Can you work these out from the model? Positions are in its coordinate system, mm. A direction names the side the tool comes from. Give positions to 0.01 mm unless a question says otherwise; leave off trailing zeros. Write each loop counter-clockwise with the first axis right and the second up, starting at its lowest first coordinate (ties: lowest second). Pieces come first, ordered by that corner, then holes.
from build123d import *

# Parameters (mm, degrees)
SKETCH_1_W          = 60
SKETCH_1_H          = 60
EXTRUDE_1_DEPTH     = 60
SKETCH_3_R          = 4
EXTRUDE_2_DEPTH     = 12
SKETCH_4_W          = 60
SKETCH_4_H          = 60
SKETCH_4_W_2        = 58
SKETCH_4_H_2        = 58
CUT_EXTRUDE_4_DEPTH = 7
FILLET_4_R          = 5
CHAMFER_1_SIZE      = 1
FILLET_6_R          = 5
SKETCH_7_W          = 28
SKETCH_7_H          = 38
EXTRUDE_3_DEPTH     = 24
SKETCH_8_W          = 44.228024
SKETCH_8_H          = 29.89004
SKETCH_8_R          = 7
CUT_EXTRUDE_5_DEPTH = 4


with BuildPart() as part:
    # 草图1 → 凸台-拉伸1 (new body)
    with BuildSketch(Plane.XY):
        Rectangle(SKETCH_1_W, SKETCH_1_H)
    extrude(amount=EXTRUDE_1_DEPTH)

    # 草图3 → 凸台-拉伸2 (add)
    with BuildSketch(Plane.XY.offset(60)):
        Circle(SKETCH_3_R)
    extrude(amount=EXTRUDE_2_DEPTH)

    # 草图4 → 切除-拉伸4 (cut)
    with BuildSketch(Plane(origin=(0, 0, 0), x_dir=(-1, 0, 0), z_dir=(0, 0, -1))):
        Rectangle(SKETCH_4_W, SKETCH_4_H)
        Rectangle(SKETCH_4_W_2, SKETCH_4_H_2, mode=Mode.SUBTRACT)
    extrude(amount=-CUT_EXTRUDE_4_DEPTH, mode=Mode.SUBTRACT)

    # 圆角4
    fillet_4_edges = [part.edges().sort_by_distance(p)[0] for p in [
        (-29, -29, 3.5),
        (29, -29, 3.5),
        (29, 29, 3.5),
        (-29, 29, 3.5),
    ]]
    fillet(fillet_4_edges, radius=FILLET_4_R)

    # 倒角1
    chamfer_1_edges = [part.edges().sort_by_distance(p)[0] for p in [
        (0, 29, 0),
        (-29, 0, 0),
        (29, 0, 0),
        (0, -29, 0),
        (27.535533906, -27.535533906, 0),
        (-27.535533906, -27.535533906, 0),
        (-27.535533906, 27.535533906, 0),
        (27.535533906, 27.535533906, 0),
    ]]
    chamfer(chamfer_1_edges, length=CHAMFER_1_SIZE)

    # 圆角6
    fillet_6_edges = [part.edges().sort_by_distance(p)[0] for p in [
        (30, -30, 33.5),
        (-30, -30, 33.5),
        (-30, 30, 33.5),
        (30, 30, 33.5),
    ]]
    fillet(fillet_6_edges, radius=FILLET_6_R)

    # 草图7 → 凸台-拉伸3 (add)
    with BuildSketch(Plane(origin=(0, 30, 0), x_dir=(1, 0, 0), z_dir=(0, 1, 0))):
        with Locations((0, -38)):
            Rectangle(SKETCH_7_W, SKETCH_7_H)
    extrude(amount=EXTRUDE_3_DEPTH)

    # 草图8 → 切除-拉伸5 (cut)
    with BuildSketch(Plane(origin=(0, 0, 19), x_dir=(-1, 0, 0), z_dir=(0, 0, -1))):
        with Locations((0, 44.94502)):
            Rectangle(SKETCH_8_W, SKETCH_8_H)
        with Locations((0, 44.94502)):
            Circle(SKETCH_8_R, mode=Mode.SUBTRACT)
    extrude(amount=-CUT_EXTRUDE_5_DEPTH, mode=Mode.SUBTRACT)


solid = part.part
(1) Imagine slicing it at C-C, the plane y = -21. Write out the boundary of the cut face in (x, z).
Returned:
outline: (-30, 7) - (-29, 7) - (-29, 1) - (-28, 0) - (28, 0) - (29, 1) - (29, 7) - (30, 7) - (30, 60) - (-30, 60) - close
(2) For faces 4 (the face through (27, -28, 4)), 5 (the face through (-0.867, -3.905, 65.916)), 6 (the face through (27, 28, 4)), which set-ups out of +Z, -Z, +X, -X, +Y, -Y let a thin tool reach every point of the face, with its end or its side?
Returned:
face 4: -Z, +X, -Y
face 5: +Z
face 6: -Z, +X, +Y
(3) Will these pins go through, and if not, where does the flat tip stop? P1, Ø4, axis at x = 6, y = 14.5, coming from the +Z side; P2, Ø12, axis at x = 7.5, z = 10, coming from the +Y side; P3, Ø3, axis at x = 4.5, y = 35, coming from the -Z side; P4, Ø4, axis at x = 16.5, y = 39, coming from the -Z side.
Returned:
P1: stops at z = 60
P2: stops at y = 30
P3: stops at z = 23
P4: passes through
(4) Imagine slicing it at D-D, the plane z = 45. Write out the boundary of the cut face in (x, y), plus the area to 3 significant figures.
Returned:
outline: (-30, -25) arc R5 ccw to (-25, -30) - (25, -30) arc R5 ccw to (30, -25) - (30, 25) arc R5 ccw to (25, 30) - (14, 30) - (14, 54) - (-14, 54) - (-14, 30) - (-25, 30) arc R5 ccw to (-30, 25) - close
area: 4,250 mm2
(5) Imagine slicing it at A-A, the plane x = 0. Write out the boundary of the cut face in (y, z).
Returned:
outline: (-30, 7) - (-29, 7) - (-29, 1) - (-28, 0) - (28, 0) - (29, 1) - (29, 7) - (30, 7) - (30, 23) - (37.95, 23) - (37.95, 19) - (51.95, 19) - (51.95, 23) - (54, 23) - (54, 57) - (30, 57) - (30, 60) - (4, 60) - (4, 72) - (-4, 72) - (-4, 60) - (-30, 60) - close
(6) If we mould it in two halves opening along Y, with no side actions, what happens to faces 1 (the face through (-14, 42, 40)), 2 (the face through (29, 28, 34)), 3 (the face through (-6.466, 42.264, 20.972))? For each: +Y half, -Y half, draft (parallel to the pull), parting line (faces both ways), or undercut.
Returned:
face 1: draft
face 2: +Y half
face 3: undercut
(7) If I drill on L1, parallel to X at y = 41.5, z = 36; L2, parallel to Z at x = -24, y = -10; L3, parallel to X at y = 21.5, z = 3.5, over which ranges is the centre line in solid material (lowest first)?
Returned:
L1: x = -14 to 14
L2: z = 0 to 60
L3: x = -29 to 29
(8) Imagine slicing it at B-B, the plane z = 10. Write out the boundary of the cut face in (x, y).
Returned:
outline: (-30, -25) arc R5 ccw to (-25, -30) - (25, -30) arc R5 ccw to (30, -25) - (30, 25) arc R5 ccw to (25, 30) - (-25, 30) arc R5 ccw to (-30, 25) - close
